Source: CAD feature listing. Evaluate the final solid. Frame: model axes, mm. Face numbers are marked on the shaded views. A direction names the side the tool comes from. Round coordinates to 2 decimals unless told otherwise and drop trailing zeros. Loops run counter-clockwise (first coordinate to the right, second up) from the corner with the lowest first, then second, coordinate; pieces in that order, holes last.
Item 1: Section query D-D on x = 1.25. Give the number of separate pieces and of enclosed holes in the cut face, then the cut area to 3 significant figures.
Item 2: Section query B-B on y = -2.5. Return loops of the section in (x, z), then the cut area to 3 significant figures.
Item 3: Section query C-C on y = -5.5. Return loops of the section in (x, z), then the cut area to 3 significant figures.
Item 4: Access query for the marked faces 4 and 5. Directions: +Z, -Z, +X, -X, +Y, -Y. A direction counts if a zero-diameter tool reaches every point of the face in a straight line with its end or side. Return the directions, or none.
Item 5: Ray query, L1, parallel to Y at x = 10.25, z = 3.75; L2, parallel to X at y = 1.25, z = 0.5; L3, parallel to Y at x = 5.5, z = 2.25. Return the intervals inside material, ascending.
Item 6: First-contact query: P1, Ø10, axis at x = 2.5, z = 2.5, coming from the -Y side; P2, Ø3, axis at y = 9, z = 3, coming from the +X side; P3, Ø2, axis at y = -3, z = 3, coming from the -X side. Flat tips, straight axial feed; report the tip coordinate or a pass-through.
Item 7: Pull-direction query (Y, two-part tool) for the marked faces 1, 2 and 3; classes: released by +Y, released by -Y, zero draft, split by the parting line, or undercut.
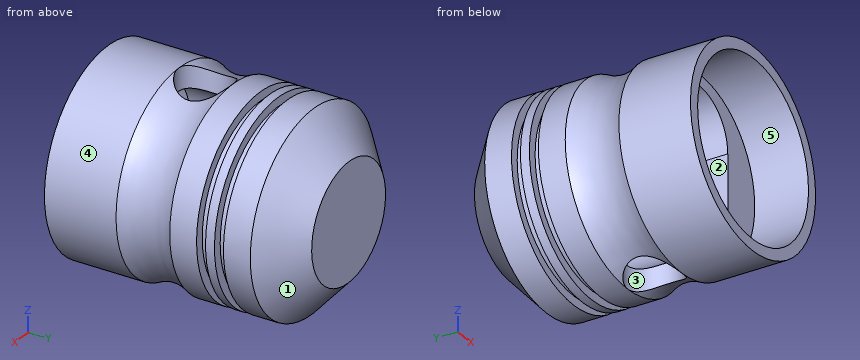
```python
from build123d import *

# Parameters (mm, degrees)
CON_ROD_SLOT_DEPTH        = 19
UNDERSIDE_BORE_SKETCH_R   = 9.75
UNDERSIDE_BORE_19_5_DEPTH = 6
WRIST_PIN_HOLE_SKETCH_R   = 3
WRIST_PIN_HOLE_6_DEPTH    = 18.500000000000004


with BuildPart() as part:
    # Piston Profile Sketch → Piston Body (revolve)
    with BuildSketch(Plane.XY, mode=Mode.PRIVATE) as piston_body_sk:
        with BuildLine():
            Line((0, -12.6437125748503), (11.000000000000002, -12.6437125748503))
            Line((11.000000000000002, -12.6437125748503), (11.000000000000002, -4.643712574850299))
            ThreePointArc((11.000000000000002, -4.643712574850299), (10.250666035204008, -1.6437125748502983), (11.000000000000002, 1.3562874251497004))
            Line((11.000000000000002, 1.3562874251497004), (11.000000000000002, 4.356287425149702))
            Line((11.000000000000002, 4.356287425149702), (10.000000000000002, 4.356287425149703))
            Line((10.000000000000002, 4.356287425149703), (10.000000000000002, 5.3562874251496995))
            Line((10.000000000000002, 5.3562874251496995), (11, 5.3562874251496995))
            Line((11, 5.3562874251496995), (11, 6.3562874251497))
            Line((11, 6.3562874251497), (10.000000000000002, 6.356287425149702))
            Line((10.000000000000002, 6.356287425149702), (10.000000000000002, 7.356287425149701))
            Line((10.000000000000002, 7.356287425149701), (11.000000000000002, 7.356287425149701))
            Line((11.000000000000002, 7.356287425149701), (11.000000000000002, 10.356287425149699))
            Line((11.000000000000002, 10.356287425149699), (6.5, 14.356287425149699))
            Line((6.5, 14.356287425149699), (-1.8e-16, 14.356287425149699))
            Line((-1.8e-16, 14.356287425149699), (0, -12.6437125748503))
        make_face()
    revolve(piston_body_sk.sketch.rotate(Axis((0, -15.6437125748503, 0), (0, 1, 0)), 90), axis=Axis((0, -15.6437125748503, 0), (0, 1, 0)))

    # Con Rod Slot Sketch → Con Rod Slot (cut)
    with BuildSketch(Plane.XZ.offset(12.6437125748503)):
        with BuildLine():
            Line((-4.999999999999999, -3.5000000000000013), (-5.000000000000002, 3.499999999999997))
            ThreePointArc((-5.000000000000002, 3.499999999999997), (-3.54e-15, 8.500000000000002), (5, 3.500000000000003))
            Line((5, 3.500000000000003), (5.000000000000003, -3.4999999999999987))
            ThreePointArc((5.000000000000003, -3.4999999999999987), (2.79e-15, -8.5), (-4.999999999999999, -3.5000000000000013))
        make_face()
    extrude(amount=-CON_ROD_SLOT_DEPTH, mode=Mode.SUBTRACT)

    # Underside Bore Sketch → Underside Bore Ø19.5 (cut)
    with BuildSketch(Plane.XZ.offset(12.6437125748503)):
        with Locations(Location((0, 0, 0), (0, 0, 270))):
            Circle(UNDERSIDE_BORE_SKETCH_R)
    extrude(amount=-UNDERSIDE_BORE_19_5_DEPTH, mode=Mode.SUBTRACT)

    # Wrist Pin Hole Sketch → Wrist Pin Hole Ø6 (cut, symmetric)
    with BuildSketch(Plane.XY):
        with Locations((0, -1.6437125748502988)):
            Circle(WRIST_PIN_HOLE_SKETCH_R)
    extrude(amount=WRIST_PIN_HOLE_6_DEPTH, both=True, mode=Mode.SUBTRACT)


solid = part.part
```
Data:
1. separate pieces: 3
1. enclosed holes: 0
1. area: 207 mm2
2. outline: (-5, -3.5) - (-5, 3.5) arc R5 cw to (-2.88, 7.59) - (-2.88, 9.9) arc R10.31 ccw to (-2.88, -9.9) - (-2.88, -7.59) arc R5 cw to start; (2.88, -9.9) arc R10.31 ccw to (2.88, 9.9) - (2.88, 7.59) arc R5 cw to (5, 3.5) - (5, -3.5) arc R5 cw to (2.88, -7.59) - close
2. area: 163 mm2
3. outline: circle Ø22 at (0, 0); hole (-5, -3.5) arc R5 ccw to (5, -3.5) - (5, 3.5) arc R5 ccw to (-5, 3.5) - close
3. area: 232 mm2
4. face 4: +Y, -Y
4. face 5: -Y
5. L1: y = -12.64 to -4.48, 1.19 to 4.36, 5.36 to 6.36, 7.36 to 10.43
5. L2: x = -10.93 to -5, 5 to 10.93
5. L3: y = -6.64 to 14.36
6. P1: stops at y = -6.64
6. P2: stops at x = 10.9
6. P3: stops at x = -10.35
7. face 1: released by +Y
7. face 2: zero draft
7. face 3: undercut
